CAD build for the part. Positions are in the model's coordinates, mm. A direction names the side the tool comes from. Give positions to 0.01 mm unless a question says otherwise; leave off trailing zeros. Loops run counter-clockwise (first coordinate to the right, second up) from the corner with the lowest first, then second, coordinate; pieces in that order, holes last. Notation, with made-up numbers: (2.25, -34.5) - (25.25, -34.5) arc R18 ccw to (25.25, -9.5) - close; hole circle Ø3 at (-28, 88). An arc over 180 degrees is marked (long way). Return JSON: item names as keys, results as strings.
from build123d import *

# Parameters (mm, degrees)
BOSS_EXTRUDE1_DEPTH = 135
CUT_EXTRUDE1_DEPTH  = 160
SKETCH3_R           = 6
CUT_EXTRUDE2_DEPTH  = 10


with BuildPart() as part:
    # Sketch1 → Boss-Extrude1 (new body)
    with BuildSketch(Plane.XY):
        Polygon((0, 0), (0, 30), (3, 30), (3, 3), (30, 3), (30, 0), align=None)
    extrude(amount=BOSS_EXTRUDE1_DEPTH)

    # Sketch2 → Cut-Extrude1 (cut)
    with BuildSketch(Plane(origin=(0, 3, 0), x_dir=(1, 0, 0), z_dir=(0, 1, 0))):
        with BuildLine():
            Line((10.658971341, -13.531915857), (20.494612748, -13.531915857))
            ThreePointArc((20.494612748, -13.531915857), (24.063483391, -17.1007865), (20.494612748, -20.669657144))
            Line((20.494612748, -20.669657144), (10.658971341, -20.669657144))
            ThreePointArc((10.658971341, -20.669657144), (7.090100697, -17.1007865), (10.658971341, -13.531915857))
        make_face()
        with BuildLine():
            Line((10.658971341, -114.317792599), (20.494612748, -114.317792599))
            ThreePointArc((20.494612748, -114.317792599), (24.161447744, -117.984627595), (20.494612748, -121.65146259))
            Line((20.494612748, -121.65146259), (10.658971341, -121.65146259))
            ThreePointArc((10.658971341, -121.65146259), (6.992136345, -117.984627595), (10.658971341, -114.317792599))
        make_face()
    extrude(amount=-CUT_EXTRUDE1_DEPTH, mode=Mode.SUBTRACT)

    # Sketch3 → Cut-Extrude2 (cut)
    with BuildSketch(Plane.ZY):
        with Locations((85, 16)):
            Circle(SKETCH3_R)
    extrude(amount=-CUT_EXTRUDE2_DEPTH, mode=Mode.SUBTRACT)


solid = part.part
1. Cut at A-A, the plane z = 85. Write the cut outline in (x, y).
Values follow:
{"outline": "(0, 0) - (30, 0) - (30, 3) - (3, 3) - (3, 10) - (0, 10) - close; (0, 22) - (3, 22) - (3, 30) - (0, 30) - close"}
2. Drill centre lines: probe 1 along Y at (x, z) = (0.8, 85); probe 2 along X at (y, z) = (15.75, 14). Where is each one in solid material? Low to high.
Values follow:
{"probe 1": "y = 0 to 10, 22 to 30", "probe 2": "x = 0 to 3"}
3. Pull direction X, two halves, no side cores. Call faces 4 (the face through (16, 2, 121.651)), 5 (the face through (1, 30, 67)), 6 (the face through (0, 15, 67)), 7 (the face through (16, 2, 114.318)): +X half, -X half, draft (parallel to the pull), parting line (faces both ways), or undercut.
Values follow:
{"face 4": "undercut", "face 5": "draft", "face 6": "-X half", "face 7": "undercut"}
4. Cut at C-C, the plane y = 16. Write the cut outline in (x, z), plus the area to 3 significant figures.
Values follow:
{"outline": "(0, 0) - (3, 0) - (3, 79) - (0, 79) - close; (0, 91) - (3, 91) - (3, 135) - (0, 135) - close", "area": "369 mm²"}
5. Cut at B-B, the plane x = 16.25. Write the cut outline in (y, z), plus the area to 3 significant figures.
Values follow:
{"outline": "(0, 0) - (3, 0) - (3, 13.53) - (0, 13.53) - close; (0, 20.67) - (3, 20.67) - (3, 114.32) - (0, 114.32) - close; (0, 121.65) - (3, 121.65) - (3, 135) - (0, 135) - close", "area": "362 mm²"}
6. Drop flat-ended pins along their axis: P1, Ø3.5, axis at x = 17.5, y = 1, coming from the -Z side; P2, Ø13.5, axis at x = 13, z = 73.5, coming from the +Y side; P3, Ø1, axis at y = 23, z = 50, coming from the +X side; P4, Ø11, axis at y = 16, z = 85, coming from the -X side. Give the stop position or say it passes through.
Values follow:
{"P1": "stops at z = 0", "P2": "stops at y = 3", "P3": "stops at x = 3", "P4": "passes through"}
7. Cut at D-D, the plane z = 116.5. Write the cut outline in (x, y), plus the area to 3 significant figures.
Values follow:
{"outline": "(0, 0) - (7.31, 0) - (7.31, 3) - (3, 3) - (3, 30) - (0, 30) - close; (23.85, 0) - (30, 0) - (30, 3) - (23.85, 3) - close", "area": "121 mm²"}
8. Which spindle directions (+Z, -Z, +X, -X, +Y, -Y) get a long thin tool onto all of the face, cutting with end or side? Do faces 1 (the face through (8.4, 2.8, 0)), 2 (the face through (3, 17, 67)), 3 (the face through (6.993, 1.521, 118.065)). Say none if no direction does.
Values follow:
{"face 1": "-Z, +X, -X, +Y, -Y", "face 2": "+Z, -Z, +X, +Y", "face 3": "+Y, -Y"}
